Can you work these out from the model? Positions are in its coordinate system, mm. A direction names the side the tool comes from. Give positions to 0.01 mm unless a question says otherwise; leave off trailing zeros. Write each loop counter-clockwise with the first axis right and the second up, starting at its lowest first coordinate (ties: lowest second). Pieces come first, ordered by that corner, then holes.
1. On a 3-axis mill with a long thin cutter (end or side, diameter ignored), from which of +Z, -Z, +X, -X, +Y, -Y can I reach the whole of each face in a straight line? I mean faces 1 (the cylindrical face through (9.51, 78.32, -0.74)), 2 (the cylindrical face through (287.48, 7.6, -0.33)), 3 (the flat face through (191, 25, 0)). Say none if no direction works.
2. Suppose I cut it at B-B (x = 137.5). Please give me the cut outline in (y, z), and give its area (3 significant figures).
3. I'm going to push flat-ended pins straight in: pin 1 (6 mm diameter, centred on x = 181.5, z = -4.5, fed in from +Y); pin 2 (5.5 mm diameter, centred on y = 25, z = 0, fed in from -X); pin 3 (6 mm diameter, centred on y = 75, z = 0, fed in from -X). Where does each tip first touch, or does it pass through?
4. Thinking about a two-plate mould opening in Y: for faces 4 (the flat face through (125, 19, 6)), 5 (the flat face through (162, 0, 0)), 6 (the cylindrical face through (9.51, 21.63, -0.44)), which applies, pulls with the +Y half, pulls with the -Y half, needs draft (parallel to the pull), parting line crosses it, or undercut?
5. If I drill on probe 1 along Y at (x, z) = (9.25, 0); probe 2 along X at (y, z) = (3.25, 0); probe 3 along Z at (x, y) = (285, 9.75), over which ranges is the centre line in solid material (lowest first)?
6. Suppose I cut it at A-A (y = 39). Please give me the cut outline in (x, z).
```python
from build123d import *

# Parameters (mm, degrees)
EXTRUDE_1_DEPTH        = 6
HOLE_WIZARD_M8_1_D     = 6.8
HOLE_WIZARD_M8_1_DEPTH = 18.75
HOLE_WIZARD_M8_1_TIP   = 2.042926105
HOLE_WIZARD_M6_1_D     = 5
HOLE_WIZARD_M6_1_DEPTH = 15
HOLE_WIZARD_M6_1_TIP   = 1.502151548


with BuildPart() as part:
    # 草图1 → 凸台-拉伸1 (new, symmetric)
    with BuildSketch(Plane.XY):
        Polygon((0, 0), (0, 90), (25, 90), (25, 65), (65, 25), (320, 25), (320, 0), align=None)
    extrude(amount=EXTRUDE_1_DEPTH, both=True)

    # M8 螺纹孔1
    with Locations(Plane(origin=(0, 75, 0), x_dir=(0, 0, -1), z_dir=(-1, 0, 0))):
        with Locations((0, 0), (0, 50)):
            Hole(HOLE_WIZARD_M8_1_D / 2, depth=HOLE_WIZARD_M8_1_DEPTH)
            with Locations((0, 0, -(HOLE_WIZARD_M8_1_DEPTH + HOLE_WIZARD_M8_1_TIP / 2))):  # 118° drill point
                Cone(0, HOLE_WIZARD_M8_1_D / 2, HOLE_WIZARD_M8_1_TIP, mode=Mode.SUBTRACT)

    # M6 螺纹孔1
    with Locations(Plane(origin=(45, 0, 0), x_dir=(0, 0, -1), z_dir=(0, -1, 0))):
        with Locations((0, 0), (0, 120), (0, 240)):
            Hole(HOLE_WIZARD_M6_1_D / 2, depth=HOLE_WIZARD_M6_1_DEPTH)
            with Locations((0, 0, -(HOLE_WIZARD_M6_1_DEPTH + HOLE_WIZARD_M6_1_TIP / 2))):  # 118° drill point
                Cone(0, HOLE_WIZARD_M6_1_D / 2, HOLE_WIZARD_M6_1_TIP, mode=Mode.SUBTRACT)


solid = part.part
```
Checks:
1. face 1: -X
1. face 2: -Y
1. face 3: +Z, -Z, +X, +Y
2. outline: (0, -6) - (25, -6) - (25, 6) - (0, 6) - close
2. area: 300 mm2
3. pin 1: stops at y = 25
3. pin 2: stops at x = 19.14
3. pin 3: stops at x = 18.99
4. face 4: needs draft
4. face 5: pulls with the -Y half
4. face 6: undercut
5. probe 1: y = 0 to 21.6, 28.4 to 71.6, 78.4 to 90
5. probe 2: x = 0 to 42.5, 47.5 to 162.5, 167.5 to 282.5, 287.5 to 320
5. probe 3: z = -6 to -2.5, 2.5 to 6
6. outline: (0, -6) - (51, -6) - (51, 6) - (0, 6) - close
